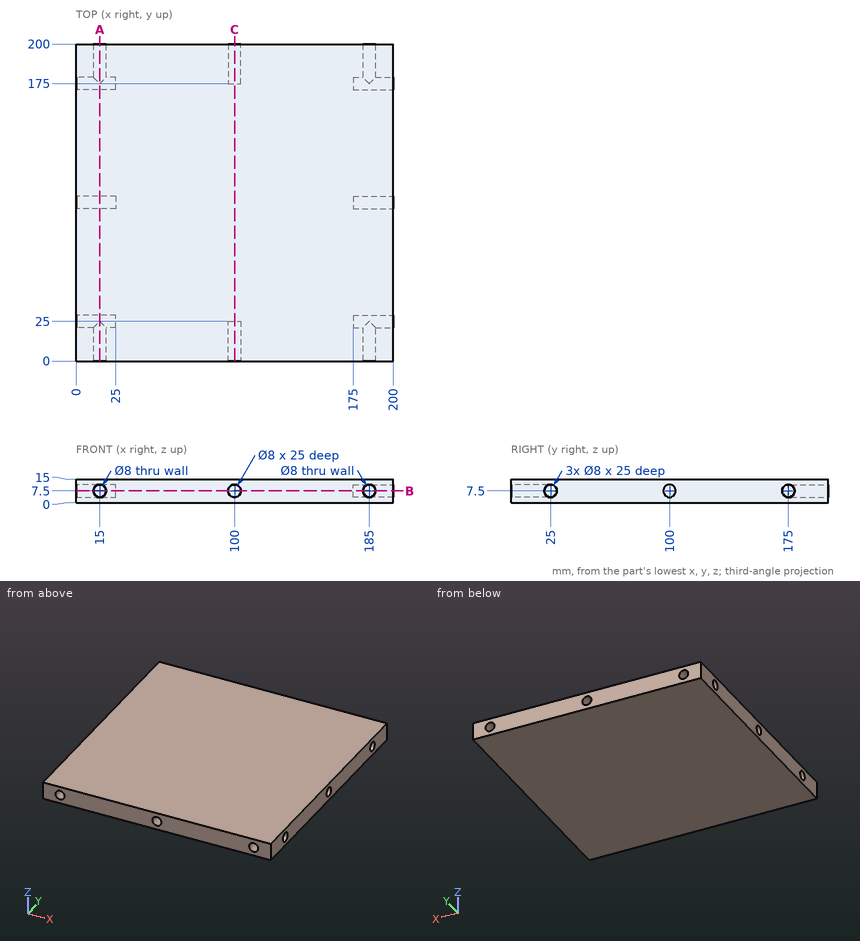
Study the drawing (mm; zero at the part's minimum x, y, z) and answer. Round coordinates to 2 decimals unless told otherwise and drop trailing zeros. Loops run counter-clockwise (first coordinate to the right, second up) from the corner with the lowest first, then second, coordinate; pieces in that order, holes last. Notation, with made-up numbers: (20.25, 27) -> (37.25, 27) arc R16 ccw to (37.25, 47) -> close; hole circle Ø4 at (-33, -32). An arc over 180 degrees is marked (long way). One line per item, written item: value.
1) A cutting plane is placed at C-C (x = 100). Determine the outline of the cut face in (y, z).
Answer list:
outline: (0, 0) -> (200, 0) -> (200, 3.5) -> (175, 3.5) -> (175, 11.5) -> (200, 11.5) -> (200, 15) -> (0, 15) -> (0, 11.5) -> (25, 11.5) -> (25, 3.5) -> (0, 3.5) -> close
2) A cutting plane is placed at A-A (x = 15). Determine the outline of the cut face in (y, z), and give its area (3 significant figures).
Answer list:
outline: (0, 0) -> (200, 0) -> (200, 3.5) -> (175, 3.5) arc R4 cw to (175, 11.5) -> (200, 11.5) -> (200, 15) -> (0, 15) -> (0, 11.5) -> (25, 11.5) arc R4 cw to (25, 3.5) -> (0, 3.5) -> close; hole circle Ø8 at (100, 7.5)
area: 2,500 mm²
3) Flat-ended cylindrical pins translate along their axes: P1, Ø7, axis at x = 100, z = 7.5, coming from the +Y side; P2, Ø5, axis at x = 100.5, z = 4.5, coming from the -Y side; P3, Ø6.5, axis at y = 175, z = 7.5, coming from the -X side; P4, Ø4, axis at y = 98.5, z = 8, coming from the +X side. Find the tip coordinate at first contact, or state that the pin passes through.
Answer list:
P1: stops at y = 175
P2: stops at y = 0
P3: stops at x = 25
P4: stops at x = 175
4) Consider L1, parallel to X at y = 194.5, z = 7.5; L2, parallel to Z at x = 19, y = 25; L3, parallel to X at y = 102.5, z = 9.5. Determine where each line is inside the solid, lowest interval first. Write a range as [from, to].
Answer list:
L1: x = [0, 11], [19, 96], [104, 181], [189, 200]
L2: z = [0, 3.5], [11.5, 15]
L3: x = [25, 175]
5) A cutting plane is placed at B-B (z = 7.5). Give the number of separate pieces and of enclosed holes in the cut face, and give its area (3 significant figures).
Answer list:
separate pieces: 5
enclosed holes: 0
area: 37,700 mm²
